The listing builds one solid part. Answer for the finished solid, in the listing's coordinates (mm). Give positions to 0.01 mm unless a question says otherwise; leave off trailing zeros. Write each loop counter-clockwise with the first axis right and the second up, starting at its lowest first coordinate (ties: lowest second). Pieces come first, ordered by that corner, then holes. Notation, with made-up numbers: M -6.75,12.25 L 14.25,12.25 A20 cw 14.25,43.25 Z; hole C -26,68.5 d1. An arc over 180 degrees is marked long. Answer as a JSON object with one key per item and string values.
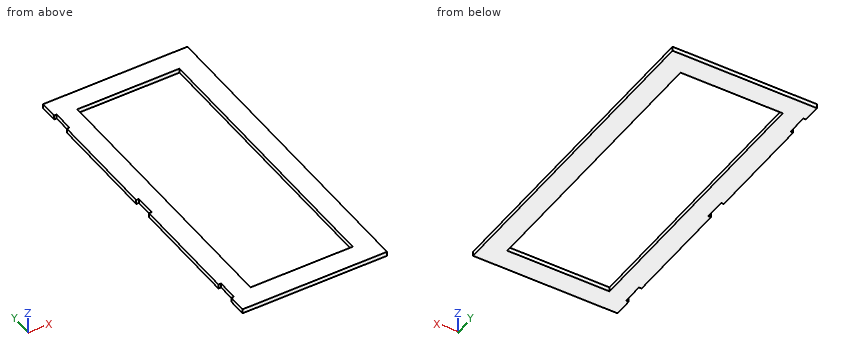
```python
from build123d import *

# Parameters (mm, degrees)
SKETCH_1_W          = 820
SKETCH_1_H          = 1820
EXTRUDE_1_DEPTH     = 25
SKETCH_2_W          = 580
SKETCH_2_H          = 1580
CUT_EXTRUDE_1_DEPTH = 999.411237918
SKETCH_3_W          = 15
SKETCH_3_H          = 117
CUT_EXTRUDE_2_DEPTH = 999.411237918


with BuildPart() as part:
    # 草图1 → 凸台-拉伸1 (new body)
    with BuildSketch(Plane.XY):
        Rectangle(SKETCH_1_W, SKETCH_1_H)
    extrude(amount=EXTRUDE_1_DEPTH)

    # 草图2 → 切除-拉伸1 (cut, through all)
    with BuildSketch(Plane.XY.offset(25)):
        Rectangle(SKETCH_2_W, SKETCH_2_H)
    extrude(amount=-CUT_EXTRUDE_1_DEPTH, mode=Mode.SUBTRACT)

    # 草图3 → 切除-拉伸2 (cut, through all)
    with BuildSketch(Plane.XY.offset(25)):
        with Locations((-402.5, -748.5)):
            Rectangle(SKETCH_3_W, SKETCH_3_H)
        with Locations((-402.5, 1.5)):
            Rectangle(SKETCH_3_W, SKETCH_3_H)
        with Locations((-402.5, 751.5)):
            Rectangle(SKETCH_3_W, SKETCH_3_H)
    extrude(amount=-CUT_EXTRUDE_2_DEPTH, mode=Mode.SUBTRACT)


solid = part.part
```
1. Consider line 1 along Y through (x, z) = (-168.5, 15); line 2 along X through (y, z) = (185, 1.5); line 3 along X through (y, z) = (-718, 8.25). Determine where each line is inside the solid, lowest interval first.
Verdict:
{"line 1": "y = -910 to -790, 790 to 910", "line 2": "x = -410 to -290, 290 to 410", "line 3": "x = -395 to -290, 290 to 410"}
2. A cutting plane is placed at C-C, the plane x = 12.5. Give the vertices of the cut face in (y, z), plus the area to 3 significant figures.
Verdict:
{"outline": "M -910,0 L -790,0 L -790,25 L -910,25 Z; M 790,0 L 910,0 L 910,25 L 790,25 Z", "area": "6,000 mm2"}
3. A cutting plane is placed at A-A, the plane z = 18. Give the vertices of the cut face in (x, y).
Verdict:
{"outline": "M -410,-910 L 410,-910 L 410,910 L -410,910 L -410,810 L -395,810 L -395,693 L -410,693 L -410,60 L -395,60 L -395,-57 L -410,-57 L -410,-690 L -395,-690 L -395,-807 L -410,-807 Z; hole M -290,-790 L 290,-790 L 290,790 L -290,790 Z"}
4. A cutting plane is placed at B-B, the plane y = 766.5. Give the vertices of the cut face in (x, z), plus the area to 4 significant figures.
Verdict:
{"outline": "M -395,0 L -290,0 L -290,25 L -395,25 Z; M 290,0 L 410,0 L 410,25 L 290,25 Z", "area": "5,625 mm2"}
5. A flat-ended cylindrical pin translates along its axis: pin 1 (7.5 mm diameter, centred on y = 12.5, z = 16.5, fed in from -X). Find the tip coordinate at first contact, or state that the pin passes through.
Verdict:
{"pin 1": "stops at x = -395"}
